Can you work these out from the drawing? Everything is in mm from the part's minimum corner. Coordinates: 2 decimals unless noted, no trailing zeros. Order: outer loops, then holes, each group sorted by start corner. A loop starts at its lowest first (then second) coordinate and runs counter-clockwise, first axis right, second up. Notation, with made-up numbers: M 53.5,17.5 L 111.5,17.5 A38 cw 111.5,55.5 Z; hole C 64,9 d6. An arc over 180 degrees is marked long. Answer as CSV lines item,"result". Start each with the question number.
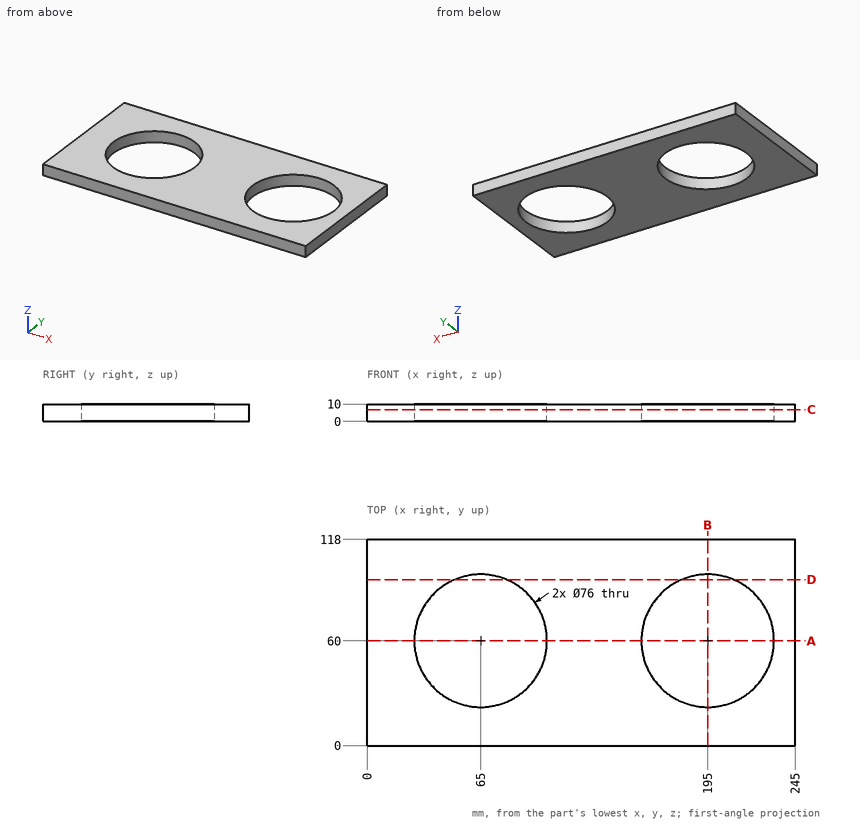
1) Suppose I cut it at B-B on x = 195. Please give me the cut outline in (y, z), plus the area to 3 significant figures.
2) Suppose I cut it at C-C on z = 6.75. Please give me the cut outline in (x, y), plus the area to 3 significant figures.
3) I need wall thicknesses on line 1 (Y direction, x = 64.5, z = 8.5); line 2 (X direction, y = 88, z = 4.5); line 3 (X direction, y = 34, z = 9.5). Which ranges of each line are inside material? Lowest first, please. Write a range as [from, to].
4) Suppose I cut it at A-A on y = 60. Please give me the cut outline in (x, z), plus the area to 3 significant figures.
5) Suppose I cut it at D-D on y = 95. Please give me the cut outline in (x, z).
Output:
1,outline,"M 0,0 L 22,0 L 22,10 L 0,10 Z; M 98,0 L 118,0 L 118,10 L 98,10 Z"
1,area,"420 mm²"
2,outline,"M 0,0 L 245,0 L 245,118 L 0,118 Z; hole C 65,60 d76; hole C 195,60 d76"
2,area,"19,800 mm²"
3,line 1,"[0, 22], [98, 118]"
3,line 2,"[0, 39.31], [90.69, 169.31], [220.69, 245]"
3,line 3,"[0, 37.29], [92.71, 167.29], [222.71, 245]"
4,outline,"M 0,0 L 27,0 L 27,10 L 0,10 Z; M 103,0 L 157,0 L 157,10 L 103,10 Z; M 233,0 L 245,0 L 245,10 L 233,10 Z"
4,area,"930 mm²"
5,outline,"M 0,0 L 50.2,0 L 50.2,10 L 0,10 Z; M 79.8,0 L 180.2,0 L 180.2,10 L 79.8,10 Z; M 209.8,0 L 245,0 L 245,10 L 209.8,10 Z"
